Here's how the part is built. I have some questions about the finished solid (model axes, mm). A direction names the side the tool comes from. Coordinates: 2 decimals unless noted, no trailing zeros. Write each loop counter-clockwise with the first axis right and the second up, starting at its lowest first coordinate (ties: lowest second). Pieces come first, ordered by that corner, then holes.
```python
from build123d import *

# Parameters (mm, degrees)
BASE_PLATE_DEPTH         = 30
PIVOT_BORE_PROFILE_R     = 20
PIVOT_BORE_DEPTH         = 30
SUPPORT_ARM_DEPTH        = 15
PIVOT_LUG_DEPTH          = 15
LUG_HOLE_PROFILE_R       = 5
LUG_HOLE_DEPTH           = 70
MOUNTING_HOLES_PROFILE_R = 5
MOUNTING_HOLES_2X_DEPTH  = 70


with BuildPart() as part:
    # Base Plate Profile → Base Plate (new body)
    with BuildSketch(Plane.XY):
        with BuildLine():
            Line((0, 0), (0, 56))
            Line((0, 56), (20, 56))
            ThreePointArc((20, 56), (30.606601718, 60.393398282), (35, 71))
            Line((35, 71), (35, 76))
            ThreePointArc((35, 76), (70, 111), (105, 76))
            Line((105, 76), (105, 71))
            ThreePointArc((105, 71), (109.393398282, 60.393398282), (120, 56))
            Line((120, 56), (125, 56))
            Line((125, 56), (140, 56))
            Line((140, 56), (140, 0))
            Line((140, 0), (0, 0))
        make_face()
    extrude(amount=BASE_PLATE_DEPTH)

    # Pivot Bore Profile → Pivot Bore (cut)
    with BuildSketch(Plane.XY.offset(30)):
        with Locations((70, 76)):
            Circle(PIVOT_BORE_PROFILE_R)
    extrude(amount=-PIVOT_BORE_DEPTH, mode=Mode.SUBTRACT)

    # Support Arm Profile → Support Arm (add)
    with BuildSketch(Plane(origin=(35, 0, 0), x_dir=(0, 0, -1), z_dir=(1, 0, 0))):
        with BuildLine():
            Line((0, 0), (0, 45))
            Line((0, 45), (45.051517306, 18.630305493))
            ThreePointArc((45.051517306, 18.630305493), (49.651503897, 7.383041358), (40, 0))
            Line((40, 0), (0, 0))
        make_face()
    extrude(amount=SUPPORT_ARM_DEPTH)

    # Pivot Lug Profile → Pivot Lug (add)
    with BuildSketch(Plane(origin=(90, 0, 0), x_dir=(0, 0, -1), z_dir=(1, 0, 0))):
        with BuildLine():
            Line((0, 0), (0, 45))
            Line((0, 45), (45.051517306, 18.630305493))
            ThreePointArc((45.051517306, 18.630305493), (49.651503897, 7.383041358), (40, 0))
            Line((40, 0), (0, 0))
        make_face()
    extrude(amount=PIVOT_LUG_DEPTH)

    # Lug Hole Profile → Lug Hole (cut)
    with BuildSketch(Plane(origin=(105, 0, 0), x_dir=(0, 0, -1), z_dir=(1, 0, 0))):
        with Locations((40, 10)):
            Circle(LUG_HOLE_PROFILE_R)
    extrude(amount=-LUG_HOLE_DEPTH, mode=Mode.SUBTRACT)

    # Mounting Holes Profile → Mounting Holes 2x (cut)
    with BuildSketch(Plane(origin=(0, 0, 0), x_dir=(-1, 0, 0), z_dir=(0, 0, -1))):
        with Locations((-124, 28)):
            Circle(MOUNTING_HOLES_PROFILE_R)
        with Locations((-16, 28)):
            Circle(MOUNTING_HOLES_PROFILE_R)
    extrude(amount=-MOUNTING_HOLES_2X_DEPTH, mode=Mode.SUBTRACT)


solid = part.part
```
1) Will these pins go through, and if not, where does the flat tip stop? pin 1 (22.5 mm diameter, centred on y = 16, z = -25.5, fed in from +X); pin 2 (10 mm diameter, centred on x = 129.5, z = 16, fed in from +Y); pin 3 (16 mm diameter, centred on x = 124, y = 28, fed in from -Z); pin 4 (13.5 mm diameter, centred on y = 31.5, z = -37, fed in from -X).
Values follow:
pin 1: stops at x = 105
pin 2: stops at y = 56
pin 3: stops at z = 0
pin 4: passes through
2) Imagine slicing it at D-D on z = -42. Please give me the cut outline in (x, y), then the cut area to 3 significant figures.
Values follow:
outline: (35, 0.2) - (50, 0.2) - (50, 5.42) - (35, 5.42) - close; (35, 14.58) - (50, 14.58) - (50, 20.42) - (35, 20.42) - close; (90, 0.2) - (105, 0.2) - (105, 5.42) - (90, 5.42) - close; (90, 14.58) - (105, 14.58) - (105, 20.42) - (90, 20.42) - close
area: 331 mm2
3) On a 3-axis mill with a long thin cutter (end or side, diameter ignored), from which of +Z, -Z, +X, -X, +Y, -Y can I reach the whole of each face in a straight line? I mean faces 1 (the face through (35, 73, 15)), 2 (the face through (50, 18, -20)), 3 (the face through (105, 74, 15)), 4 (the face through (35, 18, -20)). Say none if no direction works.
Values follow:
face 1: +Z, -Z, -X, +Y
face 2: -Z, +Y, -Y
face 3: +Z, -Z, +X, +Y
face 4: -Z, -X, +Y, -Y
4) I need wall thicknesses on probe 1 along X at (y, z) = (27.5, 21.5); probe 2 along Y at (x, z) = (124, 14); probe 3 along Y at (x, z) = (70, 9.25). Which ranges of each line are inside material? Lowest first, please.
Values follow:
probe 1: x = 0 to 11.03, 20.97 to 119.03, 128.97 to 140
probe 2: y = 0 to 23, 33 to 56
probe 3: y = 0 to 56, 96 to 111
5) We'd pull the mould along X, two halves only. Please class faces 5 (the face through (98, 10, -35)), 6 (the face through (71, 44, 0)), 7 (the face through (140, 28, 15)): pulls with the +X half, pulls with the -X half, needs draft (parallel to the pull), parting line crosses it, or undercut.
Values follow:
face 5: needs draft
face 6: undercut
face 7: pulls with the +X half
6) Imagine slicing it at B-B on z = 18. Please give me the cut outline in (x, y), then the cut area to 3 significant figures.
Values follow:
outline: (0, 0) - (140, 0) - (140, 56) - (120, 56) arc R15 cw to (105, 71) - (105, 76) arc R35 ccw to (35, 76) - (35, 71) arc R15 cw to (20, 56) - (0, 56) - close; hole circle Ø10 at (16, 28); hole circle Ø40 at (70, 76); hole circle Ø10 at (124, 28)
area: 9,850 mm2
7) Imagine slicing it at C-C on x = 70. Please give me the cut outline in (y, z).
Values follow:
outline: (0, 0) - (56, 0) - (56, 30) - (0, 30) - close; (96, 0) - (111, 0) - (111, 30) - (96, 30) - close
8) Imagine slicing it at A-A on y = 10. Please give me the cut outline in (x, z), then the cut area to 3 significant figures.
Values follow:
outline: (0, 0) - (35, 0) - (35, -35) - (50, -35) - (50, 0) - (90, 0) - (90, -35) - (105, -35) - (105, 0) - (140, 0) - (140, 30) - (0, 30) - close; (35, -50) - (50, -50) - (50, -45) - (35, -45) - close; (90, -50) - (105, -50) - (105, -45) - (90, -45) - close
area: 5,400 mm2
